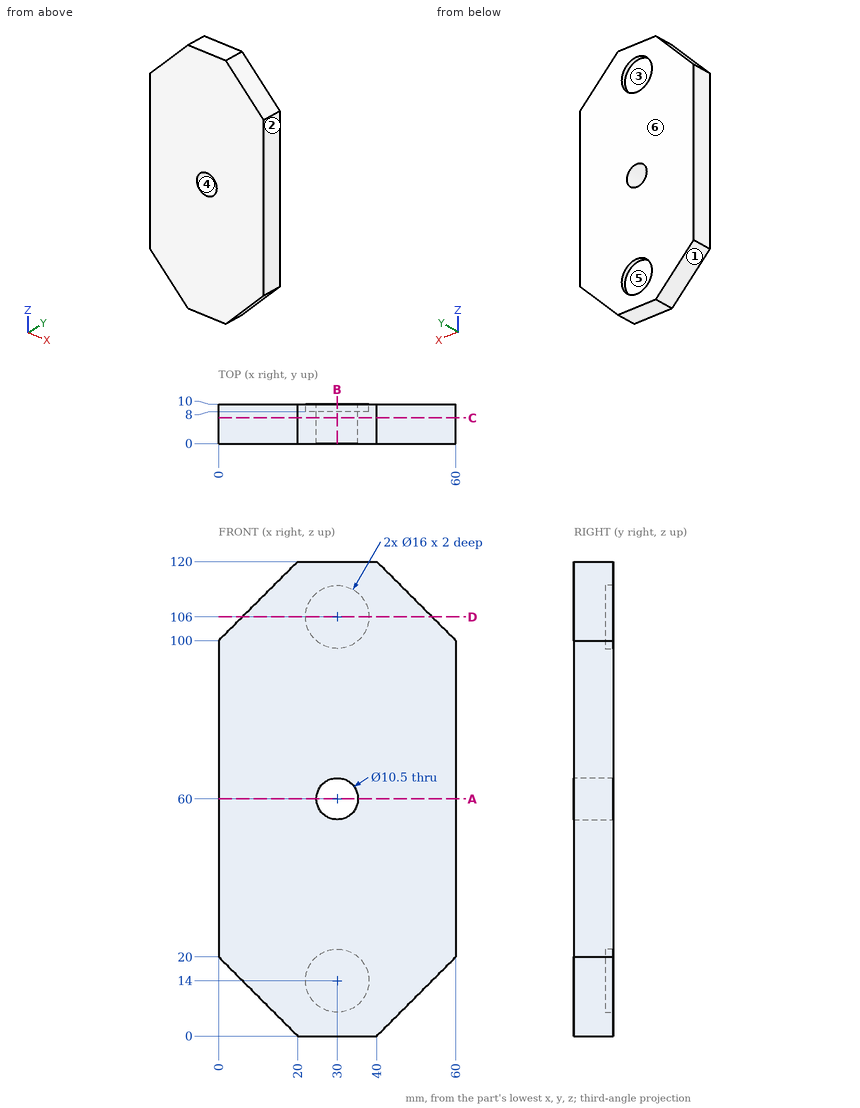
Geometry check sheet. Reference: drawing and pictorial views, mm from the part's lowest x, y, z. A direction names the side the tool comes from. Coordinates: 2 decimals unless noted, no trailing zeros. Loops run counter-clockwise (first coordinate to the right, second up) from the corner with the lowest first, then second, coordinate; pieces in that order, holes last. Notation, with made-up numbers: (11.5, 34.5) -> (59.5, 34.5) arc R30 ccw to (59.5, 73.5) -> close; hole circle Ø9 at (88, 7). An arc over 180 degrees is marked (long way). Write item = value, one per line. Start each with the question number.
1. Section check B-B on x = 30. Record the cut outline in (y, z), then the cut area to 3 significant figures.
2. Section check D-D on z = 106. Record the cut outline in (x, y).
3. Draft check along Z on the marked faces 1, 2, 3 and 4. Enter one of: released by +Z, released by -Z, zero draft, split by the parting line, or undercut.
4. Depth check by flat-ended pin: P1, Ø6, axis at x = 43.5, y = 5, coming from the -Z side; P2, Ø5, axis at x = 26.5, z = 18, coming from the +Y side; P3, Ø4, axis at x = 6.5, y = 7, coming from the -Z side. Enter the tip coordinate at first touch or a pass-through.
5. Section check C-C on y = 6.5. Record the cut outline in (x, z).
6. Material ranges on line 1 (X direction, y = 4.5, z = 57); line 2 (Z direction, x = 32, y = 5.5); line 3 (X direction, y = 3, z = 57.5), recorded low to high.
7. Tool access check on the marked faces 5 and 6. Record the directions out of +Z, -Z, +X, -X, +Y, -Y that give a thin tool (end or side, any length) a straight path to the whole face; none if there is none.
8. Section check A-A on z = 60. Record the cut outline in (x, y), then the cut area to 3 significant figures.
Responses:
q1.outline = (0, 0) -> (10, 0) -> (10, 6) -> (8, 6) -> (8, 22) -> (10, 22) -> (10, 54.75) -> (0, 54.75) -> close; (0, 65.25) -> (10, 65.25) -> (10, 98) -> (8, 98) -> (8, 114) -> (10, 114) -> (10, 120) -> (0, 120) -> close
q1.area = 1,030 mm2
q2.outline = (6, 0) -> (54, 0) -> (54, 10) -> (38, 10) -> (38, 8) -> (22, 8) -> (22, 10) -> (6, 10) -> close
q3.face_1 = released by -Z
q3.face_2 = zero draft
q3.face_3 = undercut
q3.face_4 = undercut
q4.P1 = 0.5
q4.P2 = 8
q4.P3 = 11.5
q5.outline = (0, 20) -> (20, 0) -> (40, 0) -> (60, 20) -> (60, 100) -> (40, 120) -> (20, 120) -> (0, 100) -> close; hole circle Ø10.5 at (30, 60)
q6.line_1 = 0 to 25.69, 34.31 to 60
q6.line_2 = 0 to 55.15, 64.85 to 120
q6.line_3 = 0 to 25.38, 34.62 to 60
q7.face_5 = +Y
q7.face_6 = +Z, -Z, +X, -X, +Y
q8.outline = (0, 0) -> (24.75, 0) -> (24.75, 10) -> (0, 10) -> close; (35.25, 0) -> (60, 0) -> (60, 10) -> (35.25, 10) -> close
q8.area = 495 mm2
